from build123d import *

# Parameters (mm, degrees)
CUT_EXTRUDE1_DEPTH = 1.5


with BuildPart() as part:
    # Sketch1 → Boss-Revolve (revolve)
    with BuildSketch(Plane.XY, mode=Mode.PRIVATE) as boss_revolve_sk:
        Polygon((0, 0), (6, 0), (6, 1.25), (5.25, 2), (0.268, 2), (0, 1.732), align=None)
    revolve(boss_revolve_sk.sketch.rotate(Axis((-0.277777778, 0, 0), (1, 0, 0)), 90), axis=Axis((-0.277777778, 0, 0), (1, 0, 0)))

    # Sketch2 → Cut-Extrude1 (cut)
    with BuildSketch(Plane.ZY):
        Polygon((-0.575, -0.995929214), (0.575, -0.995929214), (1.15, 0), (0.575, 0.995929214), (-0.575, 0.995929214), (-1.15, 0), align=None)
    extrude(amount=-CUT_EXTRUDE1_DEPTH, mode=Mode.SUBTRACT)

    # Sketch4 → Cut-Revolve2 (revolve, cut)
    with BuildSketch(Plane.XY, mode=Mode.PRIVATE) as cut_revolve2_sk:
        Polygon((1.5, 0.995929214), (2.075, 0), (1.5, 0), align=None)
    revolve(cut_revolve2_sk.sketch.rotate(Axis((-0.277777778, 0, 0), (1, 0, 0)), 90), axis=Axis((-0.277777778, 0, 0), (1, 0, 0)), mode=Mode.SUBTRACT)


solid = part.part
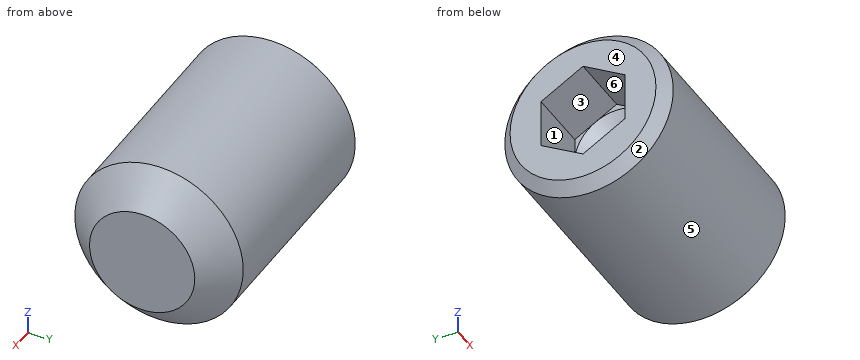
Design review of the part built by this model. Coordinates are the model's own, in mm. Face numbers are marked on the shaded views. A direction names the side the tool comes from. Round coordinates to 2 decimals unless told otherwise and drop trailing zeros. Order: outer loops, then holes, each group sorted by start corner. A loop starts at its lowest first (then second) coordinate and runs counter-clockwise, first axis right, second up.
1) Consider section A-A (x = 0.4). State the section outline as (y, z) points (3 decimals).
The answers:
outline: circle Ø4 at (0, 0); hole (-0.996, -0.575) - (0, -1.15) - (0.996, -0.575) - (0.996, 0.575) - (0, 1.15) - (-0.996, 0.575) - close
2) For L1, parallel to Y at x = 1.9, z = -0.15; L2, parallel to Y at x = 3.55, z = -1; L3, parallel to Z at x = 1.35, y = 0.5, list the stretches that pass through material, from the lowest coordinate up.
The answers:
L1: y = -1.99 to -0.26, 0.26 to 1.99
L2: y = -1.73 to 1.73
L3: z = -1.94 to -0.86, 0.86 to 1.94
3) Consider section C-C (x = 5.65). State the section outline as (y, z) points, plus the area to 3 significant figures.
The answers:
outline: circle Ø3.2 at (0, 0)
area: 8.04 mm2
4) Clearance check with a flat-ended pin moving along its axis: pin 1 Ø1.5 at (x, y) = (5.5, 1) entering from +Z. State where the tip first meets the part, or that it passes through.
The answers:
pin 1: stops at z = 1.98
5) Consider section B-B (x = 4). State the section outline as (y, z) points, plus the area to 3 significant figures.
The answers:
outline: circle Ø4 at (0, 0)
area: 12.6 mm2
6) Draft analysis for pull direction Z (two halves, no side actions). For the marked faces 1, 2, 3 and 4, state which applies: released by +Z, released by -Z, zero draft, split by the parting line, or undercut.
The answers:
face 1: undercut
face 2: split by the parting line
face 3: undercut
face 4: zero draft
7) Machinability: for the marked faces 5 and 6, which of the approach directions +Z, -Z, +X, -X, +Y, -Y give a long, thin tool a straight path to every point of the face, cutting with its end or side? Answer none if there is none.
The answers:
face 5: +X, -X
face 6: -X
